```python
from build123d import *

# Parameters (mm, degrees)
SKETCH1_W           = 110
SKETCH1_H           = 27
BOSS_EXTRUDE1_DEPTH = 8


with BuildPart() as part:
    # Sketch1 → Boss-Extrude1 (new body)
    with BuildSketch(Plane.XY):
        Rectangle(SKETCH1_W, SKETCH1_H)
    extrude(amount=BOSS_EXTRUDE1_DEPTH)

    # Sketch2 → Cut-Revolve2 (revolve, cut)
    with BuildSketch(Plane(origin=(0, 0, 0), x_dir=(1, 0, 0), z_dir=(0, 1, 0)), mode=Mode.PRIVATE) as cut_revolve2_sk:
        Polygon((-30.5, 0), (-34.5, -4), (-34.5, -8), (-38, -8), (-38, 0), align=None)
    cut_revolve2 = revolve(cut_revolve2_sk.sketch.rotate(Axis((-38, 0, 0), (0, 0, 1)), 180), axis=Axis((-38, 0, 0), (0, 0, 1)), mode=Mode.SUBTRACT)

    # Mirror1: Cut-Revolve2 across plane
    add(cut_revolve2.mirror(Plane(origin=(0, 0, 0), x_dir=(0, 0, 1), z_dir=(1, 0, 0))), mode=Mode.SUBTRACT)


solid = part.part
```
For this review, take the finished solid that the model builds, in its own axes (mm). Give positions to 0.01 mm unless a question says otherwise; leave off trailing zeros. Order: outer loops, then holes, each group sorted by start corner. A loop starts at its lowest first (then second) coordinate and runs counter-clockwise, first axis right, second up.
1) Take a section at D-D (z = 1.5). Give the boundary of the cut face in (x, y).
2) Take a section at A-A (y = 0). Give the boundary of the cut face in (x, z), then the cut area to 3 significant figures.
3) Take a section at C-C (z = 5.5). Give the boundary of the cut face in (x, y).
4) Wall thickness on line 1 (Y direction, x = 38, z = 4.85); line 2 (Y direction, x = -34, z = 1.75); line 3 (Z direction, x = 33.5, y = -0.75): over which ranges is each line inside the solid? List them lowest first.
5) Insertion check: pin 1 (8 mm diameter, centred on x = 3, y = -5.5, fed in from -Z). The pin has a flat end and moves straight along its axis. Give the tip position at first contact, or say it passes through.
6) Take a section at B-B (x = -38). Give the boundary of the cut face in (y, z), then the cut area to 3 significant figures.
7) The part is to be moulded in two halves that separate along Y. For faces 1 (the face through (-1, -13.5, 4)), 2 (the face through (34.503, -0.154, 6.028)), 3 (the face through (-1, 0, 0)), 4 (the face through (-34.503, -0.154, 6.028)), say which applies: released by +Y, released by -Y, zero draft, split by the parting line, or undercut.
Derived:
1. outline: (-55, -13.5) - (55, -13.5) - (55, 13.5) - (-55, 13.5) - close; hole circle Ø12 at (-38, 0); hole circle Ø12 at (38, 0)
2. outline: (-55, 0) - (-45.5, 0) - (-41.5, 4) - (-41.5, 8) - (-55, 8) - close; (-34.5, 4) - (-30.5, 0) - (30.5, 0) - (34.5, 4) - (34.5, 8) - (-34.5, 8) - close; (41.5, 4) - (45.5, 0) - (55, 0) - (55, 8) - (41.5, 8) - close
2. area: 736 mm2
3. outline: (-55, -13.5) - (55, -13.5) - (55, 13.5) - (-55, 13.5) - close; hole circle Ø7 at (-38, 0); hole circle Ø7 at (38, 0)
4. line 1: y = -13.5 to -3.5, 3.5 to 13.5
4. line 2: y = -13.5 to -4.13, 4.13 to 13.5
4. line 3: z = 2.94 to 8
5. pin 1: stops at z = 0
6. outline: (-13.5, 0) - (-7.5, 0) - (-3.5, 4) - (-3.5, 8) - (-13.5, 8) - close; (3.5, 4) - (7.5, 0) - (13.5, 0) - (13.5, 8) - (3.5, 8) - close
6. area: 144 mm2
7. face 1: released by -Y
7. face 2: undercut
7. face 3: zero draft
7. face 4: undercut
